Geometry check sheet. Reference: the model listing, model coordinates, mm. Give positions to 0.01 mm unless a question says otherwise; leave off trailing zeros. Write each loop counter-clockwise with the first axis right and the second up, starting at its lowest first coordinate (ties: lowest second). Pieces come first, ordered by that corner, then holes. Notation, with made-up numbers: M -38.5,-2.75 L 17.5,-2.75 A26 cw 17.5,19.25 Z; hole C 34.25,57.25 d1. An arc over 180 degrees is marked long. Write each question's results on one line, items separated by ' | '.
```python
from build123d import *

# Parameters (mm, degrees)
HEX_PROFILE_SKETCH_R = 9
HEX_NUT_BODY_DEPTH   = 5


with BuildPart() as part:
    # Hex Profile Sketch → Hex Nut Body (new, symmetric)
    with BuildSketch(Plane(origin=(0, 0, 0), x_dir=(1, 0, 0), z_dir=(0, 1, 0))):
        Polygon((14.43375673, 0), (7.216878365, 12.5), (-7.216878365, 12.5), (-14.43375673, 0), (-7.216878365, -12.5), (7.216878365, -12.5), align=None)
        with Locations(Location((0, 0, 0), (0, 0, 270))):
            Circle(HEX_PROFILE_SKETCH_R, mode=Mode.SUBTRACT)
    extrude(amount=HEX_NUT_BODY_DEPTH, both=True)

    # Chamfer Profile Sketch → Nut Chamfer Cut (revolve, cut)
    with BuildSketch(Plane.XY, mode=Mode.PRIVATE) as nut_chamfer_cut_sk:
        with BuildLine():
            Line((10.43375673, 5), (14.43375673, 5))
            Line((14.43375673, 5), (14.43375673, 1))
            ThreePointArc((14.43375673, 1), (13.262183854, 3.828427125), (10.43375673, 5))
        make_face()
    revolve(nut_chamfer_cut_sk.sketch.rotate(Axis((0, 0, 0), (0, 1, 0)), 90), axis=Axis((0, 0, 0), (0, 1, 0)), mode=Mode.SUBTRACT)


solid = part.part
```
Q1. Material ranges on probe 1 along X at (y, z) = (-1.5, -4.75); probe 2 along X at (y, z) = (1.75, 6); probe 3 along Z at (x, y) = (7.25, 1.75), recorded low to high. Write a range as [from, to].
Answer key:
probe 1: x = [-11.69, -7.64], [7.64, 11.69] | probe 2: x = [-10.97, -6.71], [6.71, 10.97] | probe 3: z = [-12.4, -5.33], [5.33, 12.4]
Q2. Section check B-B (y = -0.75). Enter the section's corners in (x, z), then the cut area to 3 significant figures.
Answer key:
outline: M -14.43,0 L -7.22,-12.5 L 7.22,-12.5 L 14.43,0 L 7.22,12.5 L -7.22,12.5 Z; hole C 0,0 d18 | area: 287 mm2
Q3. Depth check by flat-ended pin: P1, Ø1.5, axis at y = 4, z = 3, coming from the +X side; P2, Ø1.5, axis at x = 8, y = 1, coming from the -Z side. Enter the tip coordinate at first touch or a pass-through.
Answer key:
P1: stops at x = 13.12 | P2: stops at z = -12.44
Q4. Section check A-A (x = 0). Enter the section's corners in (y, z) (3 decimals).
Answer key:
outline: M -5,-12.5 L 4.425,-12.5 A4 ccw 5,-10.434 L 5,-9 L -5,-9 Z; M -5,9 L 5,9 L 5,10.434 A4 ccw 4.425,12.5 L -5,12.5 Z
Q5. Release check for a two-part mould opening along Z. For faces 1 (the face through (0, 0, 12.5)), 2 (the face through (3, -5, -9)), 3 (the face through (2.703, -0.07, 8.584)) record: released by +Z, released by -Z, zero draft, split by the parting line, or undercut.
Answer key:
face 1: released by +Z | face 2: zero draft | face 3: undercut
